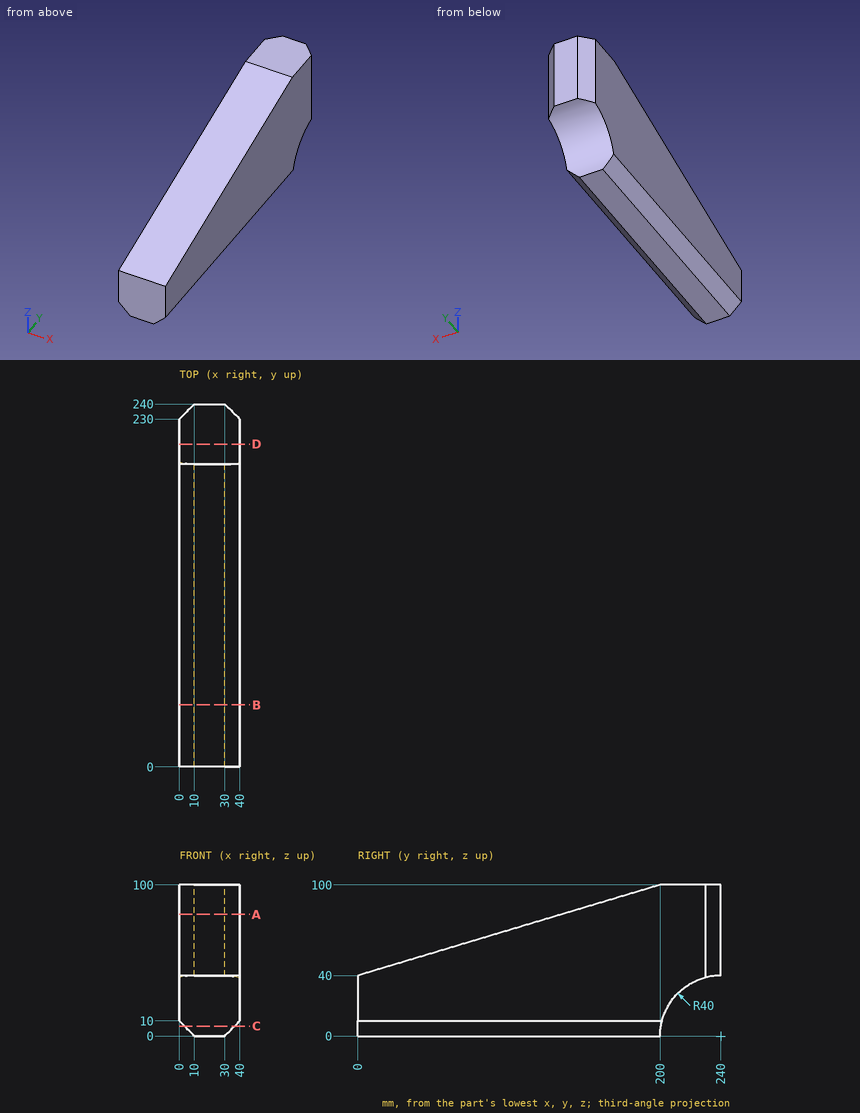
Study the drawing (mm; zero at the part's minimum x, y, z) and answer. Round coordinates to 2 decimals unless told otherwise and drop trailing zeros. Order: outer loops, then holes, each group sorted by start corner. A loop starts at its lowest first (then second) coordinate and runs counter-clockwise, first axis right, second up. Notation, with made-up numbers: (-8, -13.75) -> (20, -13.75) arc R27 cw to (20, 10.25) -> close; hole circle Ø4 at (62.25, 36.25). An arc over 180 degrees is marked (long way). Answer as CSV lines item,"result". Start each with the question number.
(1) The part is cut by section B-B (y = 41). Determine the outline of the cut face in (x, z), then the cut area to 3 significant figures.
(2) A flat-ended cylindrical pin translates along its axis: pin 1 Ø4 at (x, z) = (33.5, 66) entering from +Y. Find the tip coordinate at first contact, or state that the pin passes through.
(3) The part is cut by section C-C (z = 6.5). Determine the outline of the cut face in (x, y).
(4) The part is cut by section A-A (z = 80.5). Determine the outline of the cut face in (x, y).
(5) The part is cut by section D-D (y = 213.5). Determine the outline of the cut face in (x, z), then the cut area to 3 significant figures.
(6) Find the intervals of material crossed by probe 1 along Y at (x, z) = (33, 19); probe 2 along Y at (x, z) = (22, 24); probe 3 along Z at (x, y) = (14.5, 217.5), in increasing order. Write a range as from..to.
Evaluation:
1,outline,"(0, 10) -> (10, 0) -> (30, 0) -> (40, 10) -> (40, 52.3) -> (0, 52.3) -> close"
1,area,"1,990 mm²"
2,pin 1,"y = 238.5"
3,outline,"(3.5, 0) -> (36.5, 0) -> (36.5, 200.53) -> (3.5, 200.53) -> close"
4,outline,"(0, 135) -> (40, 135) -> (40, 230) -> (30, 240) -> (10, 240) -> (0, 230) -> close"
5,outline,"(0, 29.96) -> (40, 29.96) -> (40, 100) -> (0, 100) -> close"
5,area,"2,800 mm²"
6,probe 1,"0..204.8"
6,probe 2,"0..208"
6,probe 3,"33.07..100"
